Verification items for the finished model (mm, model axes). Face numbers are marked on the shaded views. Round coordinates to 2 decimals unless told otherwise and drop trailing zeros. Order: outer loops, then holes, each group sorted by start corner. A loop starts at its lowest first (then second) coordinate and runs counter-clockwise, first axis right, second up.
```python
from build123d import *

# Parameters (mm, degrees)
SKETCH_1_R          = 15
EXTRUDE_519_DEPTH   = 26.4
SKETCH_2_OUTSIDE_W  = 350.938
SKETCH_2_OUTSIDE_H  = 344.126
SKETCH_2_OUTSIDE_R  = 22.018695891
CUT_EXTRUDE_1_DEPTH = 38
CUT_EXTRUDE_1_DRAFT = -75
SKETCH_3_OUTSIDE_W  = 350.938
SKETCH_3_OUTSIDE_H  = 344.126
SKETCH_3_OUTSIDE_R  = 22.018695891
CUT_EXTRUDE_2_DEPTH = 38
CUT_EXTRUDE_2_DRAFT = -75


with BuildPart() as part:
    # 草图1 → Extrude 519 (new body)
    with BuildSketch(Plane.XY):
        Polygon((12.7125, 22.018695891), (-12.7125, 22.018695891), (-25.425, 0), (-12.7125, -22.018695891), (12.7125, -22.018695891), (25.425, 0), align=None)
        Circle(SKETCH_1_R, mode=Mode.SUBTRACT)
    extrude(amount=EXTRUDE_519_DEPTH)


with BuildPart() as cut_extrude_1_tool:
    # 草图2 outside → 切除-拉伸1 (with draft: the straight prism first)
    with BuildSketch(Plane(origin=(0, 0, 0), x_dir=(-1, 0, 0), z_dir=(0, 0, -1))):
        Rectangle(SKETCH_2_OUTSIDE_W, SKETCH_2_OUTSIDE_H)
        Circle(SKETCH_2_OUTSIDE_R, mode=Mode.SUBTRACT)
    extrude(amount=-CUT_EXTRUDE_1_DEPTH)
    # 切除-拉伸1: the draft: its side faces are tilted about the plane it starts from
    cut_extrude_1_sides = [cut_extrude_1_tool.faces().sort_by_distance(p)[0] for p in [
        (0, -172.063, 19),
        (-175.469, 0, 19),
        (0, 172.063, 19),
        (175.469, 0, 19),
        (22.018695891, 0, 19),
    ]]
    draft(cut_extrude_1_sides, Plane(origin=(0, 0, 0), x_dir=(-1, 0, 0), z_dir=(0, 0, -1)), CUT_EXTRUDE_1_DRAFT)


with BuildPart() as part_1:
    add(part.part)

    # 切除-拉伸1: cut by cut_extrude_1_tool
    add(cut_extrude_1_tool.part, mode=Mode.SUBTRACT)


with BuildPart() as cut_extrude_2_tool:
    # 草图3 outside → 切除-拉伸2 (with draft: the straight prism first)
    with BuildSketch(Plane.XY.offset(26.4)):
        Rectangle(SKETCH_3_OUTSIDE_W, SKETCH_3_OUTSIDE_H)
        Circle(SKETCH_3_OUTSIDE_R, mode=Mode.SUBTRACT)
    extrude(amount=-CUT_EXTRUDE_2_DEPTH)
    # 切除-拉伸2: the draft: its side faces are tilted about the plane it starts from
    cut_extrude_2_sides = [cut_extrude_2_tool.faces().sort_by_distance(p)[0] for p in [
        (0, -172.063, 7.4),
        (175.469, 0, 7.4),
        (0, 172.063, 7.4),
        (-175.469, 0, 7.4),
        (-22.018695891, 0, 7.4),
    ]]
    draft(cut_extrude_2_sides, Plane.XY.offset(26.4), CUT_EXTRUDE_2_DRAFT)


with BuildPart() as part_2:
    add(part_1.part)

    # 切除-拉伸2: cut by cut_extrude_2_tool
    add(cut_extrude_2_tool.part, mode=Mode.SUBTRACT)


solid = part_2.part
```
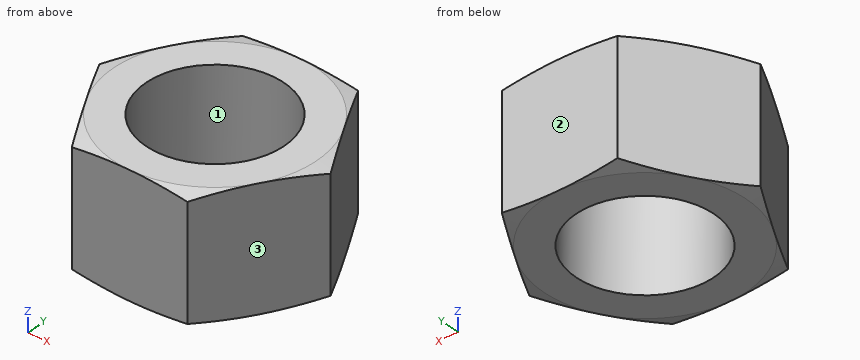
1) Sectioned sample at A-A on z = 11.5. Record the cut outline in (x, y) (1 decimal), then the cut area to 3 significant figures.
2) Go/stop test with flat-tipped pins: pin 1 Ø1 at (y, z) = (-9, 10.5) entering from +X; pin 2 Ø2 at (y, z) = (-10.5, 22) entering from -X; pin 3 Ø4 at (x, z) = (15, 13.5) entering from +Y; pin 4 Ø24 at (x, y) = (0, 0) entering from -Z. Record where each tip stops, or that it passes through.
3) Scan lines: probe 1 along Y at (x, z) = (-5, 5.75); probe 2 along X at (y, z) = (2, 17.25); probe 3 along Y at (x, z) = (4, 21). Record each from-to range of solid material in increasing order.
4) Draft check along X on the marked faces 1, 2 and 3. Enter one of: released by +X, released by -X, zero draft, split by the parting line, or undercut.
Returned:
1. outline: (-25.4, 0) - (-12.7, -22) - (12.7, -22) - (25.4, 0) - (12.7, 22) - (-12.7, 22) - close; hole circle Ø30 at (0, 0)
1. area: 973 mm2
2. pin 1: stops at x = 20.52
2. pin 2: stops at x = -19.94
2. pin 3: stops at y = 21.52
2. pin 4: passes through
3. probe 1: y = -22.02 to -14.14, 14.14 to 22.02
3. probe 2: x = -24.27 to -14.87, 14.87 to 24.27
3. probe 3: y = -22.02 to -14.46, 14.46 to 22.02
4. face 1: undercut
4. face 2: zero draft
4. face 3: released by +X
